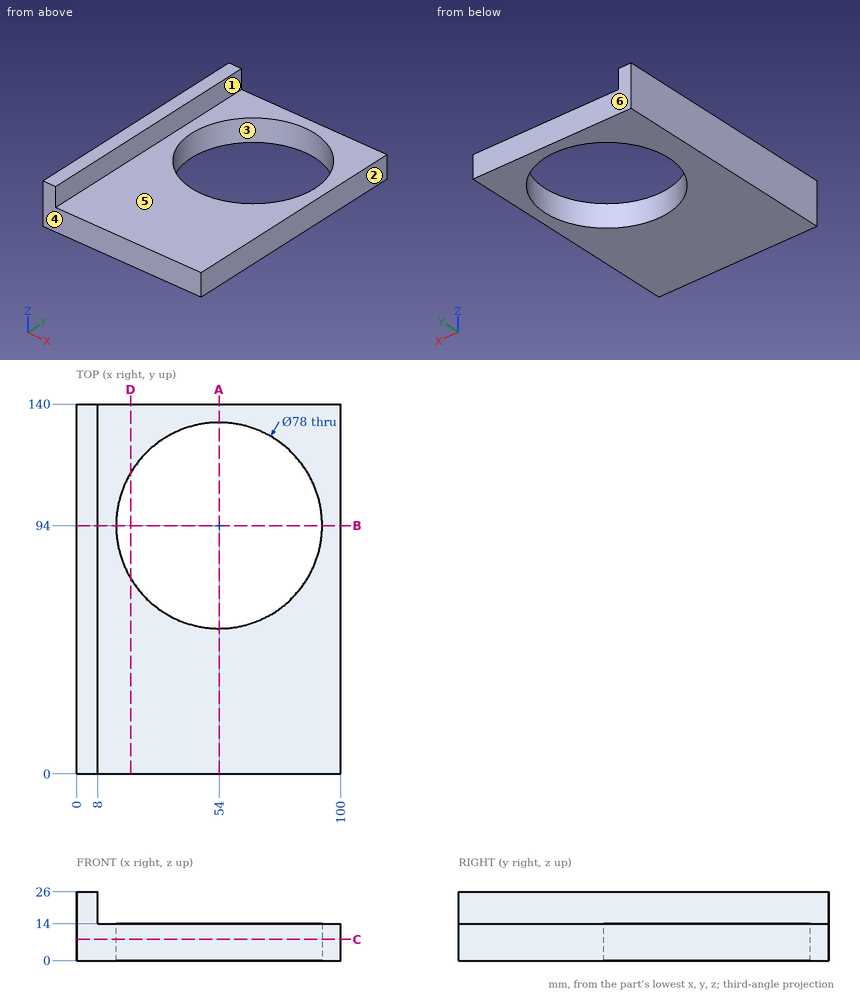
Can you work these out from the drawing? Everything is in mm from the part's minimum corner. A direction names the side the tool comes from. Coordinates: 2 decimals unless noted, no trailing zeros. Loops run counter-clockwise (first coordinate to the right, second up) from the corner with the lowest first, then second, coordinate; pieces in that order, holes last. Notation, with made-up numbers: (8, 57) - (13, 57) arc R23 cw to (13, 72) - close; hole circle Ø8 at (-25, 68.25). An arc over 180 degrees is marked (long way). Answer as CSV lines item,"result".
Q1. If I drill on L1, parallel to Y at x = 54, z = 8; L2, parallel to X at y = 44.5, z = 23.25; L3, parallel to Y at x = 47.5, z = 5, over which ranges is the centre line in solid material (lowest first)? Write a range as [from, to].
Response:
L1,"[0, 55], [133, 140]"
L2,"[0, 8]"
L3,"[0, 55.55], [132.45, 140]"
Q2. If we section it at B-B, the plane y = 94: Write out the boundary of the cut face in (x, z).
Response:
outline,"(0, 0) - (15, 0) - (15, 14) - (8, 14) - (8, 26) - (0, 26) - close; (93, 0) - (100, 0) - (100, 14) - (93, 14) - close"
Q3. For pin 1 (12 mm diameter, centred on x = 84, y = 91.5, fed in from -Z); pin 2 (3 mm diameter, centred on x = 74, y = 27.5, fed in from +Z); pin 3 (3.5 mm diameter, centred on y = 56.5, z = 20.5, fed in from +X), each with a flat end and sliding along its axis, tell me the tip position at first contact or that it passes through.
Response:
pin 1,"through"
pin 2,"z = 14"
pin 3,"x = 8"
Q4. If we section it at A-A, the plane x = 54: Write out the boundary of the cut face in (y, z), and give its area (3 significant figures).
Response:
outline,"(0, 0) - (55, 0) - (55, 14) - (0, 14) - close; (133, 0) - (140, 0) - (140, 14) - (133, 14) - close"
area,"868 mm2"
Q5. If we section it at C-C, the plane z = 8: Write out the boundary of the cut face in (x, y), and give its area (3 significant figures).
Response:
outline,"(0, 0) - (100, 0) - (100, 140) - (0, 140) - close; hole circle Ø78 at (54, 94)"
area,"9,220 mm2"
Q6. If we section it at D-D, the plane x = 20.5: Write out the boundary of the cut face in (y, z).
Response:
outline,"(0, 0) - (74.03, 0) - (74.03, 14) - (0, 14) - close; (113.97, 0) - (140, 0) - (140, 14) - (113.97, 14) - close"
Q7. For the marked faces 1 and 2, which set-ups out of +Z, -Z, +X, -X, +Y, -Y let a thin tool reach every point of the face, with its end or its side?
Response:
face 1,"+Z, +X, +Y, -Y"
face 2,"+Z, -Z, +X, +Y, -Y"
Q8. We'd pull the mould along Y, two halves only. Please class the marked faces 3, 4, 5 and 6: pulls with the +Y half, pulls with the -Y half, needs draft (parallel to the pull), parting line crosses it, or undercut.
Response:
face 3,"undercut"
face 4,"pulls with the -Y half"
face 5,"needs draft"
face 6,"pulls with the +Y half"
